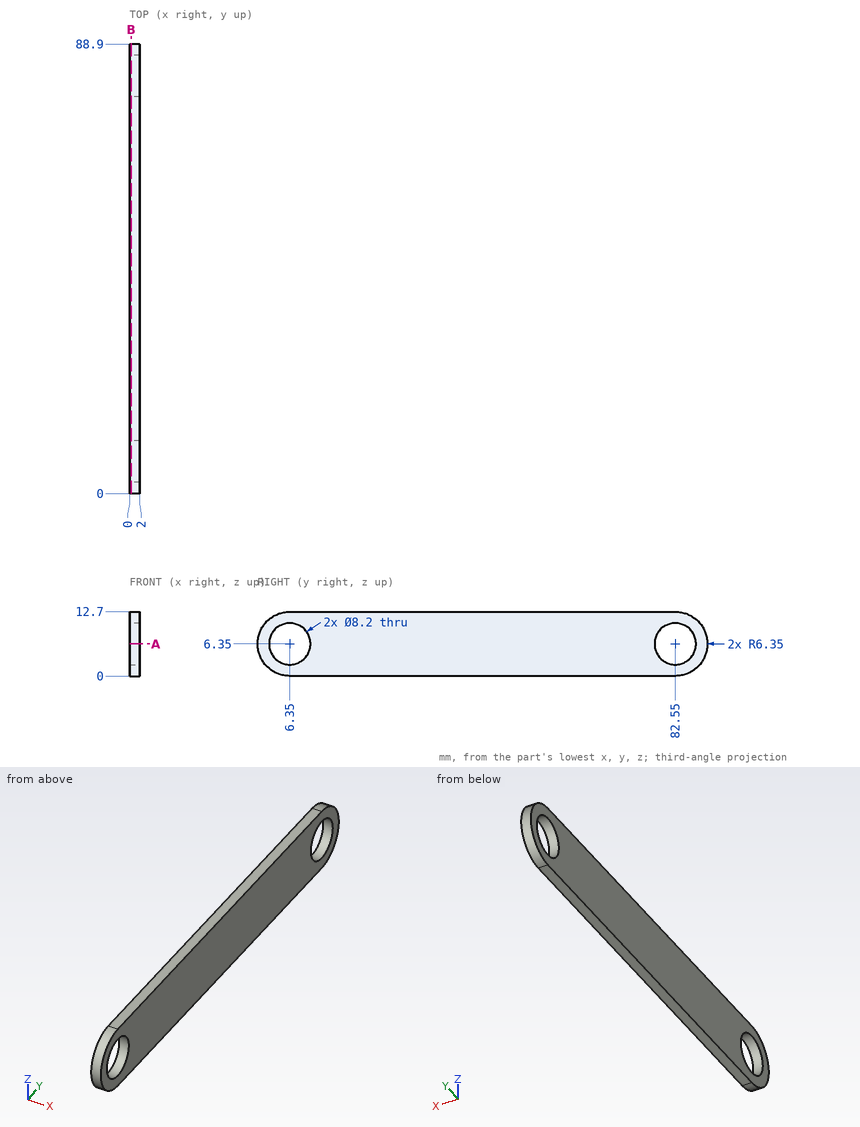
Design review of the part shown in the three views and the two pictorial views. Dimensions are in mm from the part's minimum x, y and z. Round coordinates to 2 decimals unless told otherwise and drop trailing zeros. Loops run counter-clockwise (first coordinate to the right, second up) from the corner with the lowest first, then second, coordinate; pieces in that order, holes last. Notation, with made-up numbers: M 6.25,82.5 L 15.25,82.5 A12 cw 15.25,88.5 Z; hole C 67,-2 d4. An arc over 180 degrees is marked long. Answer as a JSON object with one key per item and string values.
Item 1: Clearance check with flat-ended pins moving along their axes: P1, Ø1, axis at x = 1.5, z = 8.5, coming from the +Y side; P2, Ø7.5, axis at y = 6.35, z = 6.35, coming from the -X side; P3, Ø1, axis at x = 0.5, z = 3.5, coming from the -Y side. State where each tip first meets the part, or that it passes through.
Check sheet entries:
{"P1": "y = 88.68", "P2": "through", "P3": "y = 0.45"}
Item 2: For line 1 along Y through (x, z) = (1.1, 6.35); line 2 along Y through (x, z) = (1.05, 7.75); line 3 along Z through (x, y) = (0.65, 83), list the stretches that pass through material, from the lowest coordinate up.
Check sheet entries:
{"line 1": "0 to 2.25, 10.45 to 78.45, 86.65 to 88.9", "line 2": "0.16 to 2.5, 10.2 to 78.7, 86.4 to 88.74", "line 3": "0.02 to 2.27, 10.43 to 12.68"}
Item 3: We need section B-B, the plane x = 0.3. State the section outline as (y, z) points, and give its area (3 significant figures).
Check sheet entries:
{"outline": "M 6.35,0 L 82.55,0 A6.35 ccw 82.55,12.7 L 6.35,12.7 A6.35 ccw Z; hole C 6.35,6.35 d8.2; hole C 82.55,6.35 d8.2", "area": "989 mm2"}
Item 4: We need section A-A, the plane z = 6.35. State the section outline as (x, y) points.
Check sheet entries:
{"outline": "M 0,0 L 2,0 L 2,2.25 L 0,2.25 Z; M 0,10.45 L 2,10.45 L 2,78.45 L 0,78.45 Z; M 0,86.65 L 2,86.65 L 2,88.9 L 0,88.9 Z"}
